CAD build for the part. Positions are in the model's coordinates, mm. Face numbers are marked on the shaded views. Give positions to 0.01 mm unless a question says otherwise; leave off trailing zeros. Loops run counter-clockwise (first coordinate to the right, second up) from the corner with the lowest first, then second, coordinate; pieces in that order, holes last.
Item 1: Saw through at C-C on x = -9. Give the cut face in (y, z), plus the area to 3 significant figures.
Item 2: Saw through at B-B on y = 48. Give the cut face in (x, z).
Item 3: Probe probe 1 along Y at (x, z) = (-29.5, 11.5); probe 2 along X at (y, z) = (50.5, 9.5); probe 3 along X at (y, z) = (29.5, 36). List the from-to ranges inside material, lowest first.
Item 4: Mould opens along Y. For the marked faces 1, 2 and 3 say: released by +Y, released by -Y, zero draft, split by the parting line, or undercut.
Item 5: Drop flat-ended pins along their axis: P1, Ø3, axis at x = -126, z = 28, coming from the +Y side; P2, Ø12, axis at y = 34, z = 11, coming from the +X side; P3, Ø10, axis at y = 56, z = 26, coming from the -X side. Give the stop position or say it passes through.
Item 6: Saw through at A-A on z = 29. Give the cut face in (x, y), plus the area to 3 significant figures.
from build123d import *

# Parameters (mm, degrees)
EXTRUDE_1_DEPTH          = 43
CUT_EXTRUDE_1_DEPTH      = 470.565819802
CUT_EXTRUDE_1_DEPTH_BACK = 470.565819802


with BuildPart() as part:
    # 草图1 → 凸台-拉伸1 (new body)
    with BuildSketch(Plane.XY):
        with BuildLine():
            Line((291.578903934, -1), (-408.421096066, -1))
            ThreePointArc((-408.421096066, -1), (-457.421096066, 48), (-408.421096066, 97))
            Line((-408.421096066, 97), (-357.864757467, 97))
            Line((-357.864757467, 97), (-315.394306565, 75))
            Line((-315.394306565, 75), (-408.421096066, 75))
            ThreePointArc((-408.421096066, 75), (-435.421096066, 48), (-408.421096066, 21))
            Line((-408.421096066, 21), (291.578903934, 21))
            Line((291.578903934, 21), (291.578903934, -1))
        make_face()
    extrude(amount=EXTRUDE_1_DEPTH)

    # 草图2 → 切除-拉伸1 (cut, two sides: drawn at the far end of the back side and taken through both)
    with BuildSketch(Plane.XY.offset(43).offset(-CUT_EXTRUDE_1_DEPTH_BACK)):
        Polygon((-357.864757467, 97), (-394.373379174, 97), (-368.3426051, 75), (-315.394306565, 75), align=None)
    extrude(amount=CUT_EXTRUDE_1_DEPTH + CUT_EXTRUDE_1_DEPTH_BACK, mode=Mode.SUBTRACT)


solid = part.part
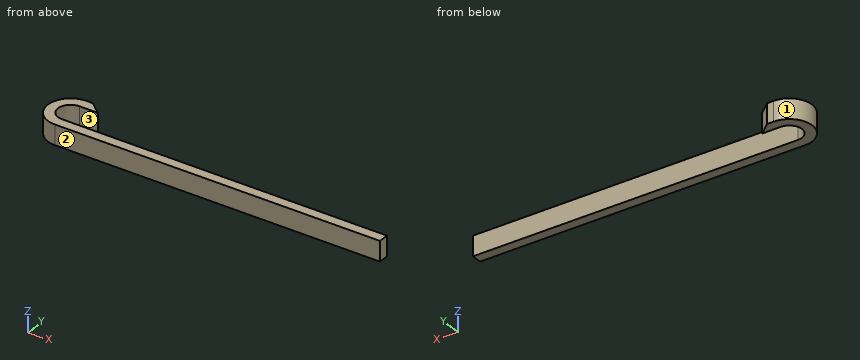
Results below:
1. outline: (-1, 0) - (21, 0) - (21, 43) - (-1, 43) - close
1. area: 946 mm2
2. outline: (-457.42, 0) - (-435.42, 0) - (-435.42, 43) - (-457.42, 43) - close
3. probe 1: y = -1 to 21
3. probe 2: x = -457.36 to -435.31
3. probe 3: x = -453.79 to -428.09
4. face 1: split by the parting line
4. face 2: released by -Y
4. face 3: undercut
5. P1: stops at y = 21
5. P2: stops at x = -426.56
5. P3: stops at x = -457.33
6. outline: (-408.42, -1) - (291.58, -1) - (291.58, 21) - (-408.42, 21) arc R27 cw to (-408.42, 75) - (-368.34, 75) - (-394.37, 97) - (-408.42, 97) arc R49 ccw to start
6. area: 18,600 mm2
